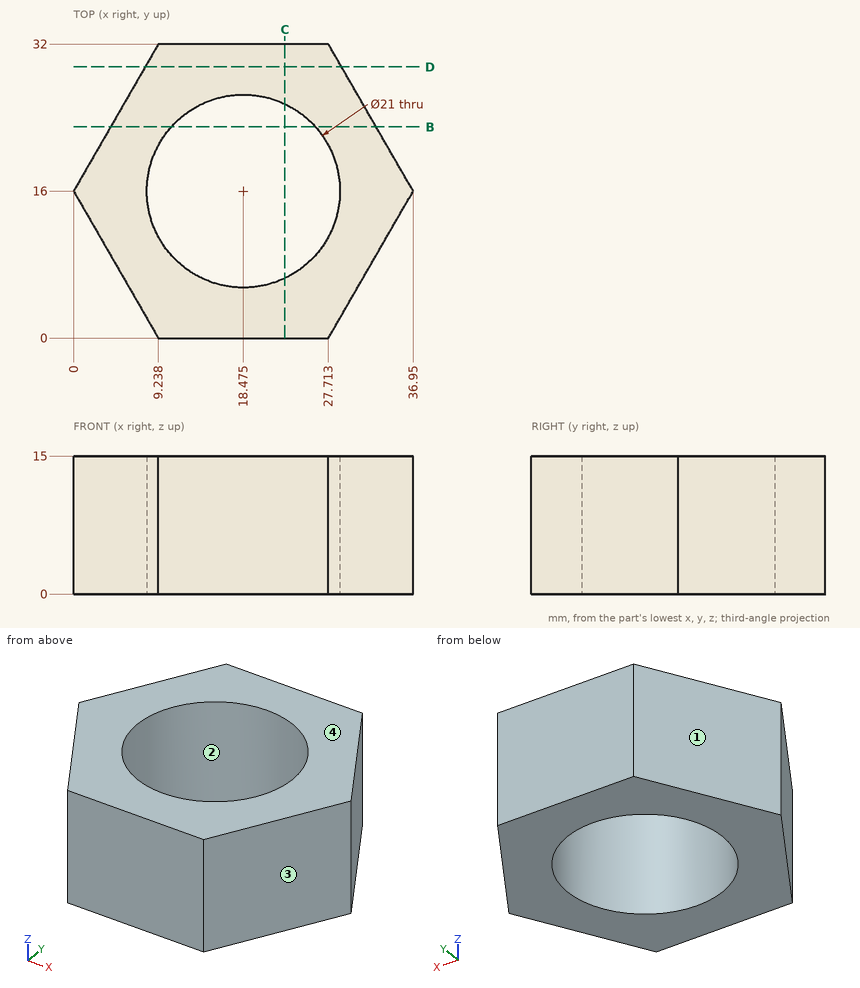
Geometry check sheet. Reference: drawing and pictorial views, mm from the part's lowest x, y, z. Round coordinates to 2 decimals unless told otherwise and drop trailing zeros. Order: outer loops, then holes, each group sorted by start corner. A loop starts at its lowest first (then second) coordinate and runs counter-clockwise, first axis right, second up. Notation, with made-up numbers: (-21.75, -2) - (4.25, -2) arc R21 cw to (4.25, 35) - close; hole circle Ø4 at (57, 88.5). An arc over 180 degrees is marked (long way). Write item = value, one per line.
Q1. Section check B-B (y = 23). Record the boundary of the cut face in (x, z), and give its area (3 significant figures).
Computed:
outline = (4.04, 0) - (10.65, 0) - (10.65, 15) - (4.04, 15) - close; (26.3, 0) - (32.91, 0) - (32.91, 15) - (26.3, 15) - close
area = 198 mm^2
Q2. Section check D-D (y = 29.5). Record the boundary of the cut face in (x, z) (1 decimal).
Computed:
outline = (7.8, 0) - (29.2, 0) - (29.2, 15) - (7.8, 15) - close
Q3. Section check C-C (x = 23). Record the boundary of the cut face in (y, z) (1 decimal), and give its area (3 significant figures).
Computed:
outline = (0, 0) - (6.5, 0) - (6.5, 15) - (0, 15) - close; (25.5, 0) - (32, 0) - (32, 15) - (25.5, 15) - close
area = 196 mm^2
Q4. Go/stop test with flat-tipped pins: pin 1 (12 mm diameter, centred on x = 28, y = 16.5, fed in from -Z); pin 2 (3 mm diameter, centred on x = 10, y = 17, fed in from +Z); pin 3 (8 mm diameter, centred on y = 19.5, z = 9.5, fed in from +X). Record where each tip stops, or that it passes through.
Computed:
pin_1 = 0
pin_2 = through
pin_3 = 36.95
Q5. Draft check along Y on the marked faces 1, 2, 3 and 4. Enter one of: pulls with the +Y half, pulls with the -Y half, needs draft (parallel to the pull), parting line crosses it, or undercut.
Computed:
face_1 = pulls with the +Y half
face_2 = undercut
face_3 = pulls with the -Y half
face_4 = needs draft
Q6. Thickness scan on line 1 along Y through (x, z) = (11, 3.75) (1 decimal); line 2 along Y through (x, z) = (11.5, 8.75); line 3 along X through (y, z) = (7.5, 11.75) (1 decimal). Record the ranges inside material, lowest first.
Computed:
line_1 = 0 to 8.6, 23.4 to 32
line_2 = 0 to 8.15, 23.85 to 32
line_3 = 4.9 to 12.3, 24.6 to 32
